```python
from build123d import *

# Parameters (mm, degrees)
SKETCH1_R           = 11
BOSS_EXTRUDE1_DEPTH = 2
SKETCH2_R           = 5
BOSS_EXTRUDE2_DEPTH = 8
SKETCH3_R           = 2.5
CUT_EXTRUDE1_DEPTH  = 19.493242009
SKETCH4_R           = 1.5
CUT_EXTRUDE2_DEPTH  = 19.493242009
SKETCH5_R           = 1.5
CUT_EXTRUDE3_DEPTH  = 7


with BuildPart() as part:
    # Sketch1 → Boss-Extrude1 (new body)
    with BuildSketch(Plane.XY):
        Circle(SKETCH1_R)
    extrude(amount=BOSS_EXTRUDE1_DEPTH)

    # Sketch2 → Boss-Extrude2 (add)
    with BuildSketch(Plane(origin=(0, 0, 0), x_dir=(-1, 0, 0), z_dir=(0, 0, -1))):
        Circle(SKETCH2_R)
    extrude(amount=BOSS_EXTRUDE2_DEPTH)

    # Sketch3 → Cut-Extrude1 (cut, through all)
    with BuildSketch(Plane(origin=(0, 0, -8), x_dir=(-1, 0, 0), z_dir=(0, 0, -1))):
        Circle(SKETCH3_R)
    extrude(amount=-CUT_EXTRUDE1_DEPTH, mode=Mode.SUBTRACT)

    # Sketch4 → Cut-Extrude2 (cut, through all)
    with BuildSketch(Plane.XY.offset(2)):
        with Locations((0, -8)):
            Circle(SKETCH4_R)
        with Locations((-8, 0)):
            Circle(SKETCH4_R)
        with Locations((0, 8)):
            Circle(SKETCH4_R)
        with Locations((8, 0)):
            Circle(SKETCH4_R)
    extrude(amount=-CUT_EXTRUDE2_DEPTH, mode=Mode.SUBTRACT)

    # Sketch5 → Cut-Extrude3 (cut, symmetric)
    with BuildSketch(Plane(origin=(0, 0, 0), x_dir=(1, 0, 0), z_dir=(0, 1, 0))):
        with Locations(Location((0, 4, 0), (0, 0, 270))):
            Circle(SKETCH5_R)
    extrude(amount=CUT_EXTRUDE3_DEPTH, both=True, mode=Mode.SUBTRACT)


solid = part.part
```
Verification items for the finished model (mm, model axes). A direction names the side the tool comes from. Round coordinates to 2 decimals unless told otherwise and drop trailing zeros. Order: outer loops, then holes, each group sorted by start corner. A loop starts at its lowest first (then second) coordinate and runs counter-clockwise, first axis right, second up. Notation, with made-up numbers: (-25.75, -37.5) - (23.25, -37.5) arc R25 ccw to (23.25, -21.5) - close; hole circle Ø9 at (0, -7). An arc over 180 degrees is marked (long way). Use CSV: the item, a comma, the result in double quotes. Start each with the question number.
1) Section check C-C, the plane z = 0.5. Record the cut outline in (x, y).
2) Thickness scan on L1, parallel to Y at x = 0, z = 0.9; L2, parallel to X at y = 2, z = 0.5; L3, parallel to Y at x = 0, z = -0.25. Record the ranges inside material, lowest first.
3) Section check B-B, the plane y = -7. Record the cut outline in (x, z).
4) Section check A-A, the plane x = 0. Record the cut outline in (y, z), plus the area to 3 significant figures.
5) Go/stop test with flat-tipped pins: P1, Ø3.5, axis at x = 0, z = -4, coming from the -Y side; P2, Ø5, axis at x = 8, y = 0, coming from the -Z side; P3, Ø6, axis at x = 0, y = 0, coming from the -Z side. Record where each tip stops, or that it passes through.
6) Mould release check, pull along Y, two halves, no side actions. Record for faces 3 (the cylindrical face through (-0.325, -9.464, 1.014)), 4 (the cylindrical face through (6.5, 0.07, 1.01)), 5 (the cylindrical face through (-4.77, 1.5, -3.94)), 6 (the flat face through (0, 3, 2)): +Y half, -Y half, draft (parallel to the pull), parting line (faces both ways), or undercut.
7) Section check D-D, the plane y = 0. Record the cut outline in (x, z).
8) Access from +Z, -Z, +X, -X, +Y, -Y to the whole of each face (thin tool, end or side, straight path). Record for faces 1 (the flat face through (5, -2, 0)), 2 (the cylindrical face through (-0.325, 6.536, 1.014)).
Answers:
1,outline,"circle Ø22 at (0, 0); hole circle Ø3 at (-8, 0); hole circle Ø5 at (0, 0); hole circle Ø3 at (0, -8); hole circle Ø3 at (0, 8); hole circle Ø3 at (8, 0)"
2,L1,"y = -11 to -9.5, -6.5 to -2.5, 2.5 to 6.5, 9.5 to 11"
2,L2,"x = -10.82 to -1.5, 1.5 to 10.82"
2,L3,"y = -5 to -2.5, 2.5 to 5"
3,outline,"(-8.49, 0) - (-1.12, 0) - (-1.12, 2) - (-8.49, 2) - close; (1.12, 0) - (8.49, 0) - (8.49, 2) - (1.12, 2) - close"
4,outline,"(-11, 0) - (-9.5, 0) - (-9.5, 2) - (-11, 2) - close; (-6.5, 0) - (-5, 0) - (-5, -2.5) - (-2.5, -2.5) - (-2.5, 2) - (-6.5, 2) - close; (-5, -8) - (-2.5, -8) - (-2.5, -5.5) - (-5, -5.5) - close; (2.5, -8) - (5, -8) - (5, -5.5) - (2.5, -5.5) - close; (2.5, -2.5) - (5, -2.5) - (5, 0) - (6.5, 0) - (6.5, 2) - (2.5, 2) - close; (9.5, 0) - (11, 0) - (11, 2) - (9.5, 2) - close"
4,area,"47.0 mm²"
5,P1,"stops at y = -5"
5,P2,"stops at z = 0"
5,P3,"stops at z = -8"
6,face 3,"undercut"
6,face 4,"undercut"
6,face 5,"parting line"
6,face 6,"draft"
7,outline,"(-11, 0) - (-9.5, 0) - (-9.5, 2) - (-11, 2) - close; (-6.5, 0) - (-5, 0) - (-5, -8) - (-2.5, -8) - (-2.5, 2) - (-6.5, 2) - close; (2.5, -8) - (5, -8) - (5, 0) - (6.5, 0) - (6.5, 2) - (2.5, 2) - close; (9.5, 0) - (11, 0) - (11, 2) - (9.5, 2) - close"
8,face 1,"-Z"
8,face 2,"+Z, -Z"
